The listing builds one solid part. Answer for the finished solid, in the listing's coordinates (mm). Face numbers are marked on the shaded views. A direction names the side the tool comes from. Give positions to 0.01 mm unless a question says otherwise; leave off trailing zeros. Write each loop counter-clockwise with the first axis right and the second up, starting at its lowest first coordinate (ties: lowest second). Pieces come first, ordered by that corner, then holes. Notation, with made-up numbers: (33.5, -30) - (67.5, -30) arc R36 cw to (67.5, 7) - close; hole circle Ø9 at (-17.75, 1.25). An arc over 180 degrees is marked (long way). Return JSON: item names as keys, results as strings.
from build123d import *

# Parameters (mm, degrees)
BOSS_EXTRUDE1_DEPTH = 6
SKETCH2_R           = 4
BOSS_EXTRUDE2_DEPTH = 20
CHAMFER1_SIZE       = 1
SCALE_1_SCALE       = 1.875


with BuildPart() as part:
    # Sketch1 → Boss-Extrude1 (new body)
    with BuildSketch(Plane.XY):
        Polygon((6.92820323, 0), (3.464101615, 6), (-3.464101615, 6), (-6.92820323, 0), (-3.464101615, -6), (3.464101615, -6), align=None)
    extrude(amount=BOSS_EXTRUDE1_DEPTH)

    # Sketch2 → Boss-Extrude2 (add)
    with BuildSketch(Plane.XY.offset(6)):
        Circle(SKETCH2_R)
    extrude(amount=BOSS_EXTRUDE2_DEPTH)

    # Chamfer1
    chamfer1_edges = [part.edges().sort_by_distance(p)[0] for p in [
        (-4, 0, 26),
    ]]
    chamfer(chamfer1_edges, length=CHAMFER1_SIZE)

    # Sketch3 → Cut-Revolve1 (revolve, cut)
    with BuildSketch(Plane(origin=(0, 0, 0), x_dir=(1, 0, 0), z_dir=(0, 1, 0)), mode=Mode.PRIVATE) as cut_revolve1_sk:
        with BuildLine():
            ThreePointArc((-6.92820323, -1), (-6.024854057, -0.306698347), (-4.92820323, 0))
            Line((-4.92820323, 0), (-8.853828921, 0.851275599))
            Line((-8.853828921, 0.851275599), (-9.311272628, -1))
            Line((-9.311272628, -1), (-6.92820323, -1))
        make_face()
        with BuildLine():
            ThreePointArc((-6.92820323, -5), (-6.024854057, -5.693301653), (-4.92820323, -6))
            Line((-4.92820323, -6), (-8.016018434, -6.744872817))
            Line((-8.016018434, -6.744872817), (-9.311272628, -5))
            Line((-9.311272628, -5), (-6.92820323, -5))
        make_face()
    revolve(cut_revolve1_sk.sketch.rotate(Axis((0, 0, 0), (0, 0, -1)), 180), axis=Axis((0, 0, 0), (0, 0, -1)), mode=Mode.SUBTRACT)


with BuildPart() as part_1:
    # Scale 1: scaled about (1e-08, -1e-08, 10.434688187)
    add(part.part.scale(SCALE_1_SCALE).moved(Location((-9e-09, 9e-09, -9.130352164))))


solid = part_1.part
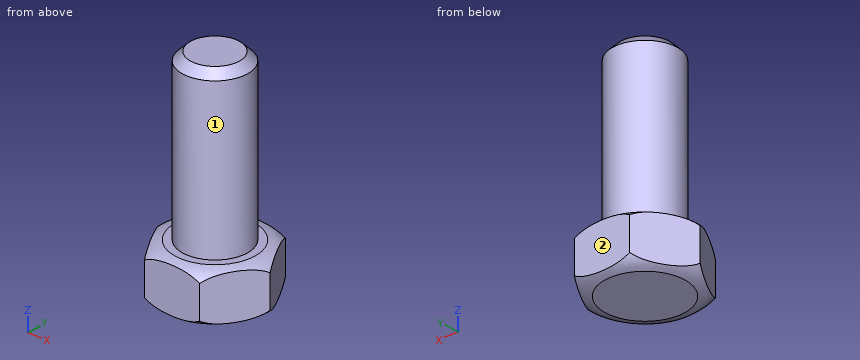
Item 1: A cutting plane is placed at A-A on z = -1.5. Determine the outline of the cut face in (x, y), then the cut area to 3 significant figures.
Answer below:
{"outline": "(-12.99, 0) - (-6.5, -11.25) - (6.5, -11.25) - (12.99, 0) - (6.5, 11.25) - (-6.5, 11.25) - close", "area": "438 mm²"}
Item 2: Flat-ended cylindrical pins translate along their axes: P1, Ø1.5, axis at y = -1.5, z = 29.5, coming from the +X side; P2, Ø10, axis at x = 9.5, z = 14.5, coming from the +Y side; P3, Ø12, axis at y = 6, z = 21.5, coming from the -X side. Find the tip coordinate at first contact, or state that the pin passes through.
Answer below:
{"P1": "stops at x = 7.46", "P2": "stops at y = 6", "P3": "stops at x = -7.5"}
Item 3: A cutting plane is placed at B-B on z = 22.5. Determine the outline of the cut face in (x, y).
Answer below:
{"outline": "circle Ø15 at (0, 0)"}
Item 4: For the marked faces 1 and 2, determine the directions among +Z, -Z, +X, -X, +Y, -Y from which every point of the face is accessible in a straight line to the end or side of a thin tool.
Answer below:
{"face 1": "+Z", "face 2": "+Z, -Z, +X, -X, +Y"}
Item 5: Consider L1, parallel to Y at x = 3.75, z = 26.5; L2, parallel to X at y = 6, z = 21; L3, parallel to X at y = 0.5, z = 4. Determine where each line is inside the solid, lowest interval first.
Answer below:
{"L1": "y = -6.5 to 6.5", "L2": "x = -4.5 to 4.5", "L3": "x = -7.48 to 7.48"}
